Here's how the part is built. I have some questions about the finished solid (model axes, mm). A direction names the side the tool comes from. Give positions to 0.01 mm unless a question says otherwise; leave off trailing zeros. Order: outer loops, then holes, each group sorted by start corner. A loop starts at its lowest first (then second) coordinate and runs counter-clockwise, first axis right, second up. Notation, with made-up numbers: (21, -32.75) - (36, -32.75) arc R7 cw to (36, -21.75) - close; hole circle Ø4 at (11.25, 72). An arc over 180 degrees is marked (long way). One line per question, with ' | ' between items.
from build123d import *

# Parameters (mm, degrees)
SKETCH_1_R      = 2.5
EXTRUDE_1_DEPTH = 3.2
SKETCH_2_R      = 4
SKETCH_2_R_2    = 2.5
EXTRUDE_2_DEPTH = 1.8
FILLET_3_R      = 0.5


with BuildPart() as part:
    # 草图1 → 凸台-拉伸1 (new body)
    with BuildSketch(Plane(origin=(0, 0, 0), x_dir=(1, 0, 0), z_dir=(0, 1, 0))):
        Polygon((4.618802154, 0), (2.309401077, 4), (-2.309401077, 4), (-4.618802154, 0), (-2.309401077, -4), (2.309401077, -4), align=None)
        with Locations(Location((0, 0, 0), (0, 0, 270))):
            Circle(SKETCH_1_R, mode=Mode.SUBTRACT)
    extrude(amount=EXTRUDE_1_DEPTH)

    # 草图2 → 凸台-拉伸2 (add)
    with BuildSketch(Plane(origin=(0, 3.2, 0), x_dir=(1, 0, 0), z_dir=(0, 1, 0))):
        with Locations(Location((0, 0, 0), (0, 0, 270))):
            Circle(SKETCH_2_R)
        with Locations(Location((0, 0, 0), (0, 0, 270))):
            Circle(SKETCH_2_R_2, mode=Mode.SUBTRACT)
    extrude(amount=EXTRUDE_2_DEPTH)

    # 圆角3
    fillet_3_edges = [part.edges().sort_by_distance(p)[0] for p in [
        (2.309401077, 1.6, 4),
        (-2.309401077, 1.6, 4),
        (-4.618802154, 1.6, 0),
        (-2.309401077, 1.6, -4),
        (2.309401077, 1.6, -4),
        (4.618802154, 1.6, 0),
        (0, 5, -4),
        (0, 5, -2.5),
    ]]
    fillet(fillet_3_edges, radius=FILLET_3_R)


solid = part.part
1) On a 3-axis mill with a long thin cutter (end or side, diameter ignored), from which of +Z, -Z, +X, -X, +Y, -Y can I reach the whole of each face in a straight line? I mean faces 4 (the face through (2.1, 3.2, 3.6)), 5 (the face through (-2.1, 3.2, -3.6)), 6 (the face through (-3.905, 3.841, -0.867)), 7 (the face through (-2.1, 3.2, 3.6)). Say none if no direction works.
Model answer:
face 4: +Z, +X, +Y | face 5: -Z, -X, +Y | face 6: +Y | face 7: +Z, -X, +Y
2) I want a section at B-B (y = 0.6). List the corners of the cut face in (x, z) for me, plus the area to 3 significant figures.
Model answer:
outline: (-4.47, -0.25) - (-2.45, -3.75) arc R0.5 ccw to (-2.02, -4) - (2.02, -4) arc R0.5 ccw to (2.45, -3.75) - (4.47, -0.25) arc R0.5 ccw to (4.47, 0.25) - (2.45, 3.75) arc R0.5 ccw to (2.02, 4) - (-2.02, 4) arc R0.5 ccw to (-2.45, 3.75) - (-4.47, 0.25) arc R0.5 ccw to start; hole circle Ø5 at (0, 0) | area: 35.7 mm2
3) I want a section at A-A (z = 0). List the corners of the cut face in (x, y) for me, plus the area to 3 significant figures.
Model answer:
outline: (-4.54, 0) - (-2.5, 0) - (-2.5, 4.5) arc R0.5 ccw to (-3, 5) - (-3.5, 5) arc R0.5 ccw to (-4, 4.5) - (-4, 3.2) - (-4.54, 3.2) - close; (2.5, 0) - (4.54, 0) - (4.54, 3.2) - (4, 3.2) - (4, 4.5) arc R0.5 ccw to (3.5, 5) - (3, 5) arc R0.5 ccw to (2.5, 4.5) - close | area: 18.3 mm2
4) Please list where these lines run through material, in increasing order: L1, parallel to X at y = 1.2, z = 0; L2, parallel to X at y = 4.35, z = -0.5; L3, parallel to Z at x = 0.75, y = 1.4.
Model answer:
L1: x = -4.54 to -2.5, 2.5 to 4.54 | L2: x = -3.97 to -2.45, 2.45 to 3.97 | L3: z = -4 to -2.38, 2.38 to 4
5) Thinking about a two-plate mould opening in X: for faces 1 (the face through (2.1, 3.2, -3.6)), 2 (the face through (-2.44, 2.22, -0.54)), 3 (the face through (3.45, 1.578, 2.025)), which applies, +X half, -X half, draft (parallel to the pull), parting line (faces both ways), or undercut?
Model answer:
face 1: draft | face 2: undercut | face 3: +X half
6) I want a section at C-C (y = 4.2). List the corners of the cut face in (x, z) for me.
Model answer:
outline: circle Ø8 at (0, 0); hole circle Ø5 at (0, 0)
7) I'm going to push a flat-ended pin straight in: P1, Ø1, axis at y = 1, z = 2, coming from the -X side. Where does the tip first touch, or does it pass through?
Model answer:
P1: stops at x = -3.75
